from build123d import *
from OCP.BRepFilletAPI import BRepFilletAPI_MakeChamfer

# Parameters (mm, degrees)
SKETCH_1_R            = 20
SKETCH_1_R_2          = 14
EXTRUDE_1_DEPTH       = 95
SKETCH_3_W            = 2.5
SKETCH_3_H            = 11
SKETCH_3_W_2          = 1.25
SKETCH_3_H_2          = 1.7
SKETCH_4_R            = 14
SKETCH_4_R_2          = 11
EXTRUDE_2_DEPTH       = 14
CHAMFER_1_SIZE        = 0.5
HOLE_WIZARD_4_0_4_3_D = 4
SKETCH_7_W            = 2
SKETCH_7_H            = 10
CUT_EXTRUDE_1_DEPTH   = 10
CHAMFER_2_SIZE        = 2
CHAMFER_2_SIZE2       = 3.464101615


with BuildPart() as part:
    # 草图1 → 凸台-拉伸1 (new body)
    with BuildSketch(Plane(origin=(0, 0, 0), x_dir=(1, 0, 0), z_dir=(0, 1, 0))):
        with Locations(Location((0, 0, 0), (0, 0, 270))):
            Circle(SKETCH_1_R)
        with Locations(Location((0, 0, 0), (0, 0, 270))):
            Circle(SKETCH_1_R_2, mode=Mode.SUBTRACT)
    extrude(amount=EXTRUDE_1_DEPTH)

    # 草图3 → 切除-旋转1 (revolve, cut)
    with BuildSketch(Plane.XY, mode=Mode.PRIVATE) as cut_revolve_1_sk:
        with Locations((18.75, 68)):
            Rectangle(SKETCH_3_W, SKETCH_3_H)
        with Locations((19.375, 89.65)):
            Rectangle(SKETCH_3_W_2, SKETCH_3_H_2)
    revolve(cut_revolve_1_sk.sketch.rotate(Axis((0, 0, 0), (0, 1, 0)), 90), axis=Axis((0, 0, 0), (0, 1, 0)), mode=Mode.SUBTRACT)

    # 草图4 → 凸台-拉伸2 (add)
    with BuildSketch(Plane.XZ):
        with Locations(Location((0, 0, 0), (0, 0, 270))):
            Circle(SKETCH_4_R)
        with Locations(Location((0, 0, 0), (0, 0, 270))):
            Circle(SKETCH_4_R_2, mode=Mode.SUBTRACT)
    extrude(amount=-EXTRUDE_2_DEPTH)

    # 倒角1
    chamfer_1_edges = [part.edges().sort_by_distance(p)[0] for p in [
        (0, 0, -20),
        (0, 95, -20),
    ]]
    chamfer(chamfer_1_edges, length=CHAMFER_1_SIZE)

    # Ø4.0 (4) 直径孔3 (through all)
    with Locations(Plane(origin=(20, 8, 0), x_dir=(0, 0, 1), z_dir=(1, 0, 0))):
        with Locations((0, 0)):
            Hole(HOLE_WIZARD_4_0_4_3_D / 2)

    # 草图7 → 切除-拉伸1 (cut, symmetric)
    with BuildSketch(Plane.XY):
        with Locations((-19, 35)):
            Rectangle(SKETCH_7_W, SKETCH_7_H)
    extrude(amount=CUT_EXTRUDE_1_DEPTH, both=True, mode=Mode.SUBTRACT)

    # 倒角2: one chamfer whose edges measure the first distance from different faces: ONE call of the kernel's chamfer builder (chamfer() names one face for all edges)
    chamfer_2_edges_1 = [part.edges().sort_by_distance(p)[0] for p in [
        (0, 0, 11),
    ]]
    chamfer_2_side_1 = [part.faces().sort_by_distance(p)[0] for p in [
        (0, 0, -18.948456711),
    ]]
    chamfer_2_edges_2 = [part.edges().sort_by_distance(p)[0] for p in [
        (0, 95, -14),
    ]]
    chamfer_2_side_2 = [part.faces().sort_by_distance(p)[0] for p in [
        (0, 95, -18.948456711),
    ]]
    chamfer_2 = BRepFilletAPI_MakeChamfer(part.part.solid().wrapped)
    for e in chamfer_2_edges_1:
        chamfer_2.Add(CHAMFER_2_SIZE, CHAMFER_2_SIZE2, e.wrapped, chamfer_2_side_1[0].wrapped)  # the first distance lies on this face
    for e in chamfer_2_edges_2:
        chamfer_2.Add(CHAMFER_2_SIZE, CHAMFER_2_SIZE2, e.wrapped, chamfer_2_side_2[0].wrapped)  # the first distance lies on this face
    add(Compound.cast(chamfer_2.Shape()), mode=Mode.REPLACE)


solid = part.part
The listing builds one solid part. Answer for the finished solid, in the listing's coordinates (mm). A direction names the side the tool comes from. Give positions to 0.01 mm unless a question says otherwise; leave off trailing zeros. Loops run counter-clockwise (first coordinate to the right, second up) from the corner with the lowest first, then second, coordinate; pieces in that order, holes last.
Item 1: Find the intervals of material crossed by line 1 along Y through (x, z) = (-13.5, 14); line 2 along Y through (x, z) = (16.75, 0); line 3 along Z through (x, y) = (0.5, 89.5), in increasing order.
Derived:
line 1: y = 0 to 62.5, 73.5 to 88.8, 90.5 to 95
line 2: y = 0 to 6, 10 to 95
line 3: z = -18.74 to -13.99, 13.99 to 18.74
Item 2: Each of these flat-tipped pins is pushed along its axis until it touches: pin 1 Ø2.5 at (y, z) = (8, 0) entering from -X; pin 2 Ø8 at (y, z) = (33.5, 0.5) entering from -X; pin 3 Ø0.6 at (x, z) = (-19.5, -1) entering from +Y; pin 4 Ø8 at (y, z) = (67.5, 6) entering from -X. Where does it stop, or does it pass through?
Derived:
pin 1: passes through
pin 2: stops at x = -20
pin 3: stops at y = 95
pin 4: stops at x = -17.39
Item 3: A cutting plane is placed at B-B (z = 0). Give the number of separate pieces and of enclosed holes in the cut face, then the cut area to 3 significant figures.
Derived:
separate pieces: 4
enclosed holes: 0
area: 1,060 mm2
Item 4: A cutting plane is placed at C-C (y = 28). Give the vertices of the cut face in (x, z), then the cut area to 3 significant figures.
Derived:
outline: circle Ø40 at (0, 0); hole circle Ø28 at (0, 0)
area: 641 mm2
Item 5: A cutting plane is placed at A-A (y = 9). Give the vertices of the cut face in (x, z).
Derived:
outline: (-19.92, -1.73) arc R20 ccw to (19.92, -1.73) - (10.86, -1.73) arc R11 cw to (-10.86, -1.73) - close; (-19.92, 1.73) - (-10.86, 1.73) arc R11 cw to (10.86, 1.73) - (19.92, 1.73) arc R20 ccw to start
Item 6: A tool of negligible diameter and unlimited length cuts with its end or side. For faces 4 (the flat face through (18, 73.5, 0)), 5 (the flat face through (-9.3, 14, -6.2)), 6 (the flat face through (-19, 30, 0)), from which of +Z, -Z, +X, -X, +Y, -Y can it reach the whole face along a straight path? Write none if from no direction.
Derived:
face 4: none
face 5: +Y
face 6: +Z, -Z, -X
Item 7: Determine the mould class of faces 1 (the flat face through (-18, 35, 0)), 2 (the cylindrical face through (15, 6, 0)), 3 (the cylindrical face through (16.864, 31.066, 10.752)) for opening direction Z: +Z half, -Z half, draft (parallel to the pull), parting line (faces both ways), or undercut.
Derived:
face 1: draft
face 2: undercut
face 3: parting line
